Input: part model. Units: mm. Frame: model coordinates. A direction names the side the tool comes from. Coordinates: 2 decimals unless noted, no trailing zeros. Loops run counter-clockwise (first coordinate to the right, second up) from the corner with the lowest first, then second, coordinate; pieces in that order, holes last.
Item 1: Section C-C on z = 4.5. Return loops of the section in (x, y).
Item 2: Section A-A on x = 36. Return loops of the section in (y, z).
Item 3: Reachability of faces 1 (the flat face through (3, -27.5, 12)), 2 (the cylindrical face through (255.494, 0.561, 12.325)) from +Z, -Z, +X, -X, +Y, -Y: full face, straight path, thin tool, end or side. Return the list, or none.
Item 4: Section B-B on y = 17. Return loops of the section in (x, z), and give its area (3 significant figures).
Item 5: Contact query for flat-ended pins moving along their axis: P1, Ø12, axis at y = 5, z = 9, coming from the -X side; P2, Ø4, axis at y = -21, z = 21.5, coming from the -X side; P3, Ø1, axis at y = 18, z = 5.5, coming from the +X side. Output: stop coordinate, or through.
Item 6: Ray query, line 1 along Y through (x, z) = (143, 11.5); line 2 along X through (y, z) = (-0.5, 16.25); line 3 along X through (y, z) = (17, 17). Return the intervals inside material, ascending.
Item 7: Pull-direction query (X, two-part tool) for faces 3 (the flat face through (-3, 25.5, 12)), 4 (the flat face through (-3, 27.5, 12)), 5 (the cylindrical face through (-257.493, -0.605, 12.325)); classes: released by +X, released by -X, zero draft, split by the parting line, or undercut.
```python
from build123d import *

# Parameters (mm, degrees)
EXTRUDE_1_DEPTH = 25


with BuildPart() as part:
    # 草图1 → 拉伸-薄壁1 (new body)
    with BuildSketch(Plane.XY):
        with BuildLine():
            Line((230, -27.5), (-230, -27.5))
            ThreePointArc((-230, -27.5), (-257.5, 0), (-230, 27.5))
            Line((-230, 27.5), (230, 27.5))
            ThreePointArc((230, 27.5), (257.5, 0), (230, -27.5))
        make_face()
        with BuildLine():
            Line((230, -25.5), (-230, -25.5))
            ThreePointArc((-230, -25.5), (-255.5, 0), (-230, 25.5))
            Line((-230, 25.5), (230, 25.5))
            ThreePointArc((230, 25.5), (255.5, 0), (230, -25.5))
        make_face(mode=Mode.SUBTRACT)
    extrude(amount=EXTRUDE_1_DEPTH)


solid = part.part
```
Results found:
1. outline: (-230, -27.5) - (230, -27.5) arc R27.5 ccw to (230, 27.5) - (-230, 27.5) arc R27.5 ccw to start; hole (-230, -25.5) - (230, -25.5) arc R25.5 ccw to (230, 25.5) - (-230, 25.5) arc R25.5 ccw to start
2. outline: (-27.5, 0) - (-25.5, 0) - (-25.5, 25) - (-27.5, 25) - close; (25.5, 0) - (27.5, 0) - (27.5, 25) - (25.5, 25) - close
3. face 1: +Z, -Z, +X, -X, -Y
3. face 2: +Z, -Z
4. outline: (-251.62, 0) - (-249.01, 0) - (-249.01, 25) - (-251.62, 25) - close; (249.01, 0) - (251.62, 0) - (251.62, 25) - (249.01, 25) - close
4. area: 130 mm2
5. P1: stops at x = -257.5
5. P2: stops at x = -249.88
5. P3: stops at x = 251.21
6. line 1: y = -27.5 to -25.5, 25.5 to 27.5
6. line 2: x = -257.5 to -255.5, 255.5 to 257.5
6. line 3: x = -251.62 to -249.01, 249.01 to 251.62
7. face 3: undercut
7. face 4: zero draft
7. face 5: released by -X
